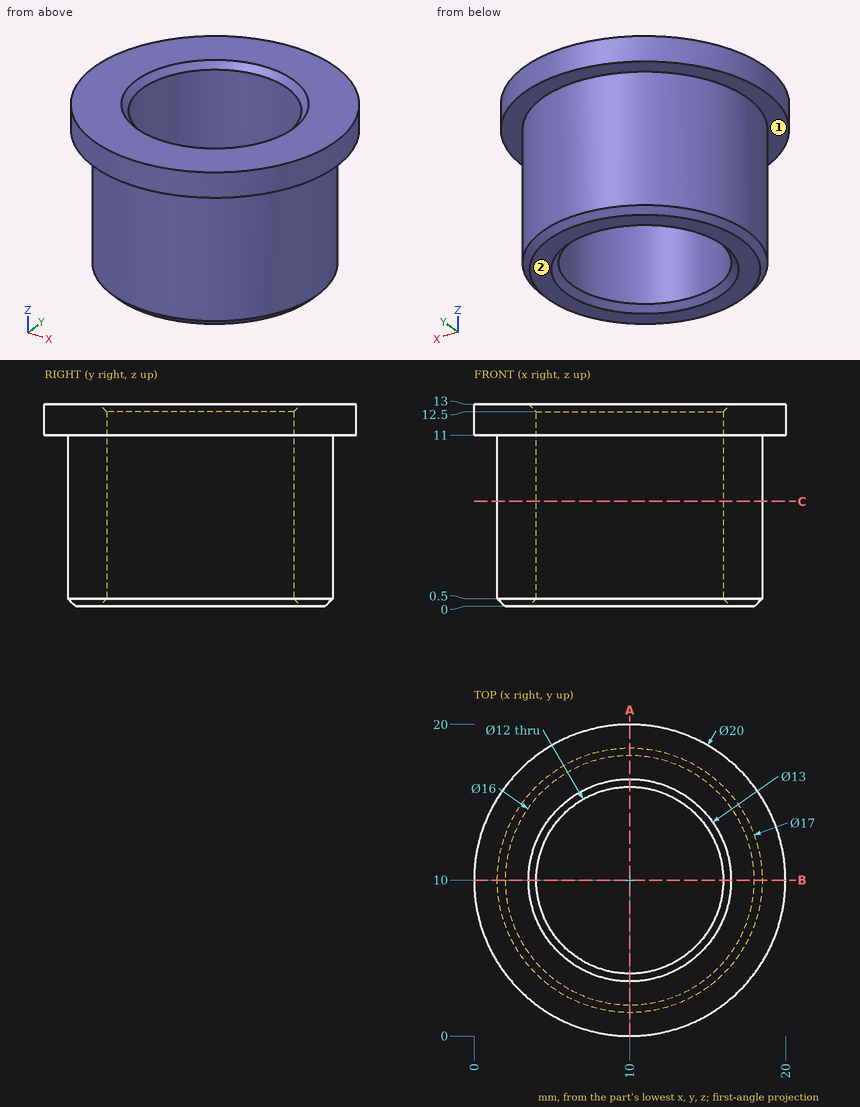
Input: dimensioned drawing with shaded views. Units: mm. Origin: part minimum x, y, z. A direction names the side the tool comes from. Coordinates: 2 decimals unless noted, no trailing zeros. Write each loop counter-clockwise with the first axis right and the second up, starting at its lowest first coordinate (ties: lowest second). Pieces come first, ordered by that corner, then holes. Notation, with made-up numbers: (-15, 19.5) -> (7, 19.5) arc R28 ccw to (7, 58.5) -> close; hole circle Ø2 at (-2, 3). An arc over 180 degrees is marked (long way). Return JSON: item names as keys, results as strings. Group by question number.
1) Section query C-C, the plane z = 6.75. Return loops of the section in (x, y).
2) Contact query for flat-ended pins moving along their axis: P1, Ø1.5, axis at x = 8, z = 10.5, coming from the +Y side; P2, Ø5, axis at y = 10.5, z = 2, coming from the +X side; P3, Ø1.5, axis at y = 3.5, z = 4.5, coming from the +X side. Output: stop coordinate, or through.
3) Section query A-A, the plane x = 10. Return loops of the section in (y, z).
4) Ray query, line 1 along Y through (x, z) = (10, 9.5); line 2 along X through (y, z) = (6.5, 11.5); line 3 along Y through (x, z) = (8.25, 3.75). Return the intervals inside material, ascending.
5) Set-up query: the marked faces 1 and 2. Return all of +Z, -Z, +X, -X, +Y, -Y with unobstructed straight access to the full face (end or side cutting, diameter ignored); none if empty.
From the geometry:
{
 "1": {"outline": "circle Ø17 at (10, 10); hole circle Ø12 at (10, 10)"},
 "2": {"P1": "y = 19.9", "P2": "x = 18.5", "P3": "x = 16.26"},
 "3": {"outline": "(0, 11) -> (1.5, 11) -> (1.5, 0.5) -> (2, 0) -> (3.5, 0) -> (4, 0.5) -> (4, 12.5) -> (3.5, 13) -> (0, 13) -> close; (16, 0.5) -> (16.5, 0) -> (18, 0) -> (18.5, 0.5) -> (18.5, 11) -> (20, 11) -> (20, 13) -> (16.5, 13) -> (16, 12.5) -> close"},
 "4": {"line 1": "1.5 to 4, 16 to 18.5", "line 2": "0.63 to 5.13, 14.87 to 19.37", "line 3": "1.68 to 4.26, 15.74 to 18.32"},
 "5": {"face 1": "-Z", "face 2": "-Z, +X, -X, +Y, -Y"}
}
